Work out the finished part from the listing and answer in its coordinate system (mm). A direction names the side the tool comes from. Give positions to 0.01 mm unless a question says otherwise; leave off trailing zeros. Loops run counter-clockwise (first coordinate to the right, second up) from the corner with the lowest first, then second, coordinate; pieces in that order, holes last. Notation, with made-up numbers: M -27.75,49 L -17.75,49 A16 ccw -17.75,73 Z; hole C -5.5,5 d5. An arc over 180 degrees is marked long. Use a Markdown table: item, result.
```python
from build123d import *

# Parameters (mm, degrees)
SKETCH2_R          = 16.5
CUT_EXTRUDE1_DEPTH = 20
SKETCH3_R          = 9
CUT_EXTRUDE2_DEPTH = 20


with BuildPart() as part:
    # Sketch1 → Revolve1 (revolve)
    with BuildSketch(Plane.XY, mode=Mode.PRIVATE) as revolve1_sk:
        Polygon((-19.588974855, 112), (-19.588974855, 182.5), (-4.588974855, 182.5), (-4.588974855, 131.5), (21.411025145, 131.5), (21.411025145, 112), align=None)
    revolve(revolve1_sk.sketch.rotate(Axis((-91.426499033, 0, 0), (1, 0, 0)), 90), axis=Axis((-91.426499033, 0, 0), (1, 0, 0)))

    # Sketch2 → Cut-Extrude1 (cut)
    with BuildSketch(Plane.ZY.offset(19.588974855)):
        with Locations((61.229349178, 147.820725202)):
            Circle(SKETCH2_R)
        with Locations((147.820725202, 61.229349178)):
            Circle(SKETCH2_R)
        with Locations((147.820725202, -61.229349178)):
            Circle(SKETCH2_R)
        with Locations((61.229349178, -147.820725202)):
            Circle(SKETCH2_R)
        with Locations((-61.229349178, -147.820725202)):
            Circle(SKETCH2_R)
        with Locations((-147.820725202, -61.229349178)):
            Circle(SKETCH2_R)
        with Locations((-147.820725202, 61.229349178)):
            Circle(SKETCH2_R)
        with Locations((-61.229349178, 147.820725202)):
            Circle(SKETCH2_R)
    extrude(amount=-CUT_EXTRUDE1_DEPTH, mode=Mode.SUBTRACT)

    # Sketch3 → Cut-Extrude2 (cut)
    with BuildSketch(Plane.ZY.offset(19.588974855)):
        with Locations((0, 160)):
            Circle(SKETCH3_R)
        with Locations((160, 0)):
            Circle(SKETCH3_R)
        with Locations((0, -160)):
            Circle(SKETCH3_R)
        with Locations((-160, 0)):
            Circle(SKETCH3_R)
    extrude(amount=-CUT_EXTRUDE2_DEPTH, mode=Mode.SUBTRACT)


solid = part.part
```
(1) A cutting plane is placed at D-D (y = 136). Write down the section's boundary in (x, z).
Entries:
| item | result |
|---|---|
| outline | M -19.59,-121.7 L -4.59,-121.7 L -4.59,-72.74 L -19.59,-72.74 Z; M -19.59,-49.72 L -4.59,-49.72 L -4.59,49.72 L -19.59,49.72 Z; M -19.59,72.74 L -4.59,72.74 L -4.59,121.7 L -19.59,121.7 Z |
(2) A cutting plane is placed at C-C (x = 12). Write down the section's boundary in (y, z), and give its area (3 significant figures).
Entries:
| item | result |
|---|---|
| outline | C 0,0 d263; hole C 0,0 d224 |
| area | 14,900 mm² |
(3) Consider probe 1 along Z at (x, y) = (-5.5, 146); probe 2 along Z at (x, y) = (-12.5, -49); probe 3 along Y at (x, z) = (-14.5, 160). Determine where each line is inside the solid, lowest interval first. Write a range as [from, to].
Entries:
| item | result |
|---|---|
| probe 1 | z = [-109.5, -77.63], [-44.83, 44.83], [77.63, 109.5] |
| probe 2 | z = [-175.8, -158.9], [-136.74, -100.71], [100.71, 136.74], [158.9, 175.8] |
| probe 3 | y = [-87.79, -72.36], [-50.1, -9], [9, 50.1], [72.36, 87.79] |
(4) Given P1, Ø12, axis at x = -8.5, y = -65.5, coming from the -Z side; P2, Ø10, axis at x = -7.5, z = -88, coming from the -Y side; P3, Ø5, axis at y = 100.5, z = 130, coming from the +X side, each flat-ended and moving along its own axis, determine where each tip first touches the part or whether it passes through.
Entries:
| item | result |
|---|---|
| P1 | stops at z = -172.53 |
| P2 | stops at y = -162.53 |
| P3 | stops at x = -4.59 |
(5) The mould has two halves that part along Z. Classify faces 3 (the flat face through (-4.589, -55, -123)), 4 (the cylindrical face through (-12.194, -60.504, 131.337)), 5 (the cylindrical face through (-11.98, -54.82, 174.07)): released by +Z, released by -Z, zero draft, split by the parting line, or undercut.
Entries:
| item | result |
|---|---|
| face 3 | zero draft |
| face 4 | undercut |
| face 5 | split by the parting line |
(6) A cutting plane is placed at A-A (y = 0). Write down the section's boundary in (x, z), and give its area (3 significant figures).
Entries:
| item | result |
|---|---|
| outline | M -19.59,-182.5 L -4.59,-182.5 L -4.59,-169 L -19.59,-169 Z; M -19.59,-151 L -4.59,-151 L -4.59,-131.5 L 21.41,-131.5 L 21.41,-112 L -19.59,-112 Z; M -19.59,112 L 21.41,112 L 21.41,131.5 L -4.59,131.5 L -4.59,151 L -19.59,151 Z; M -19.59,169 L -4.59,169 L -4.59,182.5 L -19.59,182.5 Z |
| area | 2,590 mm² |
(7) Which of the six approach directions +Z, -Z, +X, -X, +Y, -Y give full straight-line access (tool end or side, diameter ignored) to faces 1 (the cylindrical face through (8.593, -110.881, 70.694)), 2 (the cylindrical face through (-12.194, 131.713, 57.652))?
Entries:
| item | result |
|---|---|
| face 1 | +X |
| face 2 | +X, -X |
